```python
from build123d import *

# Parameters (mm, degrees)
SKETCH2_R          = 11
CUT_EXTRUDE1_DEPTH = 15
CIRPATTERN1_COUNT  = 4
CUT_EXTRUDE2_DEPTH = 15
CHAMFER1_SIZE      = 1
CHAMFER1_SIZE2     = 0.577350269
CHAMFER2_SIZE      = 1
CHAMFER2_SIZE2     = 0.577350269
CHAMFER3_SIZE      = 1
CHAMFER3_SIZE2     = 0.577350269


with BuildPart() as part:
    # Sketch1 → Revolve1 (revolve)
    with BuildSketch(Plane.XY, mode=Mode.PRIVATE) as revolve1_sk:
        Polygon((-36.947368421, 131.5), (-3.947368421, 131.5), (-3.947368421, 178), (11.052631579, 178), (11.052631579, 112), (-36.947368421, 112), align=None)
    revolve(revolve1_sk.sketch.rotate(Axis((-77.413533835, 0, 0), (1, 0, 0)), 90), axis=Axis((-77.413533835, 0, 0), (1, 0, 0)))

    # Sketch2 → Cut-Extrude1 (cut)
    with BuildSketch(Plane(origin=(11.052631579, 0, 0), x_dir=(0, 0, -1), z_dir=(1, 0, 0))):
        with Locations((111.722871427, 111.722871427)):
            Circle(SKETCH2_R)
    cut_extrude1 = extrude(amount=-CUT_EXTRUDE1_DEPTH, mode=Mode.SUBTRACT)

    # CirPattern1: Cut-Extrude1 ×4 about axis
    cirpattern1_axis = Axis((0, 0, 0), (1, 0, 0))
    for i in range(1, CIRPATTERN1_COUNT):
        add(cut_extrude1.rotate(cirpattern1_axis, i * 360 / CIRPATTERN1_COUNT), mode=Mode.SUBTRACT)

    # Sketch3 → Cut-Extrude2 (cut)
    with BuildSketch(Plane(origin=(11.052631579, 0, 0), x_dir=(0, 0, -1), z_dir=(1, 0, 0))):
        with BuildLine():
            Line((-95.833188406, 150), (95.833188406, 150))
            ThreePointArc((95.833188406, 150), (0, 178), (-95.833188406, 150))
        make_face()
        with BuildLine():
            Line((-150, 95.833188406), (-150, -95.833188406))
            ThreePointArc((-150, -95.833188406), (-178, 0), (-150, 95.833188406))
        make_face()
        with BuildLine():
            Line((-95.833188406, -150), (95.833188406, -150))
            ThreePointArc((95.833188406, -150), (0, -178), (-95.833188406, -150))
        make_face()
        with BuildLine():
            Line((150, 95.833188406), (150, -95.833188406))
            ThreePointArc((150, -95.833188406), (178, 0), (150, 95.833188406))
        make_face()
    extrude(amount=-CUT_EXTRUDE2_DEPTH, mode=Mode.SUBTRACT)

    # Chamfer1
    chamfer1_edges = [part.edges().sort_by_distance(p)[0] for p in [
        (11.052631579, 0, -112),
    ]]
    chamfer1_side = [part.faces().sort_by_distance(p)[0] for p in [
        (-12.947368421, 0, -112),
    ]]
    chamfer(chamfer1_edges, length=CHAMFER1_SIZE, length2=CHAMFER1_SIZE2, reference=chamfer1_side[0])

    # Chamfer2
    chamfer2_edges = [part.edges().sort_by_distance(p)[0] for p in [
        (-36.947368421, 0, -112),
    ]]
    chamfer2_side = [part.faces().sort_by_distance(p)[0] for p in [
        (-36.947368421, 0, -115.719381669),
    ]]
    chamfer(chamfer2_edges, length=CHAMFER2_SIZE, length2=CHAMFER2_SIZE2, reference=chamfer2_side[0])

    # Chamfer3
    chamfer3_edges = [part.edges().sort_by_distance(p)[0] for p in [
        (-36.947368421, 0, -131.5),
    ]]
    chamfer3_side = [part.faces().sort_by_distance(p)[0] for p in [
        (-20.447368421, 0, -131.5),
    ]]
    chamfer(chamfer3_edges, length=CHAMFER3_SIZE, length2=CHAMFER3_SIZE2, reference=chamfer3_side[0])


solid = part.part
```
Source: CAD feature listing. Evaluate the final solid. Frame: model axes, mm. A direction names the side the tool comes from. Coordinates: 2 decimals unless noted, no trailing zeros. Order: outer loops, then holes, each group sorted by start corner. A loop starts at its lowest first (then second) coordinate and runs counter-clockwise, first axis right, second up. Notation, with made-up numbers: (79.5, 26.25) - (106.5, 26.25) arc R31 cw to (106.5, 50.25) - close; hole circle Ø4 at (11.25, 59). An arc over 180 degrees is marked (long way). One line per item, written item: value.
1) Mould query, pull axis Y, two halves, no side actions, for faces 1 (the face through (-13.484, 99.363, 51.681)), 2 (the face through (4, 1, 150)), 3 (the face through (3.66, 126.25, 125.48)). Classes: released by +Y, released by -Y, zero draft, split by the parting line, or undercut.
Computed values:
face 1: undercut
face 2: zero draft
face 3: released by +Y
2) Cut plane C-C on x = -26. Output: boundary loops of the cut face in (y, z), plus the area to 3 significant figures.
Computed values:
outline: circle Ø263 at (0, 0); hole circle Ø224 at (0, 0)
area: 14,900 mm^2
3) Ray query, line 1 (X direction, y = 133, z = -76.5); line 2 (Y direction, x = -3, z = 16); line 3 (Y direction, x = -13, z = -98.5). Return the intervals inside material, ascending. Write a range as [from, to].
Computed values:
line 1: x = [-3.95, 11.05]
line 2: y = [-150, -110.85], [110.85, 150]
line 3: y = [-87.12, -53.31], [53.31, 87.12]
4) Reachability of faces 4 (the face through (3.66, -110.29, -122.63)), 5 (the face through (-3.947, -2, 135)) from +Z, -Z, +X, -X, +Y, -Y: full face, straight path, thin tool, end or side. Return the list, or none.
Computed values:
face 4: +X, -X
face 5: -X
5) Contact query for flat-ended pins moving along their axis: pin 1 (5 mm diameter, centred on y = -99, z = 47, fed in from -X); pin 2 (6 mm diameter, centred on x = -8.5, y = -72, fed in from +Z); pin 3 (1 mm diameter, centred on x = -17.5, z = 117.5, fed in from -Y); pin 4 (13 mm diameter, centred on y = 111.72, z = 111.72, fed in from -X). Output: stop coordinate, or through.
Computed values:
pin 1: stops at x = -36.42
pin 2: stops at z = 111.94
pin 3: stops at y = -60.03
pin 4: passes through
6) Cut plane A-A on y = 0. Output: boundary loops of the cut face in (x, z), plus the area to 3 significant figures.
Computed values:
outline: (-36.95, -130.92) - (-35.95, -131.5) - (-3.95, -131.5) - (-3.95, -150) - (11.05, -150) - (11.05, -112.58) - (10.05, -112) - (-36.37, -112) - (-36.95, -113) - close; (-36.95, 113) - (-36.37, 112) - (10.05, 112) - (11.05, 112.58) - (11.05, 150) - (-3.95, 150) - (-3.95, 131.5) - (-35.95, 131.5) - (-36.95, 130.92) - close
area: 2,430 mm^2
